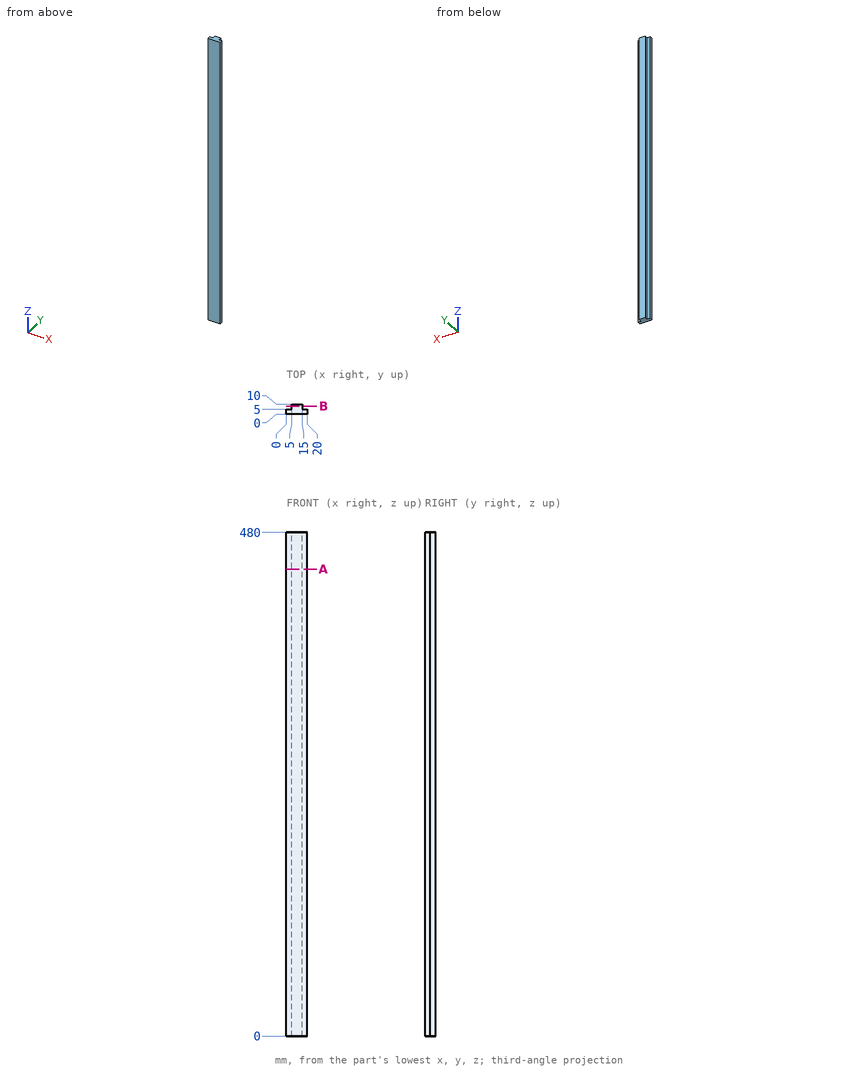
The drawing under review shows one solid part. Ordinate dimensions are in mm from its lowest x, y, z. Give positions to 0.01 mm unless a question says otherwise; leave off trailing zeros. Order: outer loops, then holes, each group sorted by start corner. A loop starts at its lowest first (then second) coordinate and runs counter-clockwise, first axis right, second up. Notation, with made-up numbers: (26.25, -14.5) - (55.25, -14.5) arc R28 cw to (55.25, 8.5) - close; hole circle Ø10 at (59.25, 50). An arc over 180 degrees is marked (long way). Answer as a JSON object with one key per item and string values. Group by question number.
Item 1: Wall thickness on line 1 along Y through (x, z) = (15.75, 396); line 2 along X through (y, z) = (5.5, 82.5): over which ranges is each line inside the solid? List them lowest first.
Item 2: Take a section at B-B on y = 8. Give the boundary of the cut face in (x, z).
Item 3: Clearance check with flat-ended pins moving along their axes: pin 1 Ø3 at (y, z) = (2.5, 319) entering from -X; pin 2 Ø1.5 at (y, z) = (8, 257) entering from -X; pin 3 Ø1.5 at (y, z) = (7, 210.5) entering from +X; pin 4 Ø1.5 at (x, z) = (18.5, 348.5) entering from +Y. State where each tip first meets the part, or that it passes through.
Item 4: Take a section at A-A on z = 445. Give the boundary of the cut face in (x, y).
Reported:
{
 "1": {"line 1": "0 to 5", "line 2": "5 to 15"},
 "2": {"outline": "(5, 0) - (15, 0) - (15, 480) - (5, 480) - close"},
 "3": {"pin 1": "x = 0", "pin 2": "x = 5", "pin 3": "x = 15", "pin 4": "y = 5"},
 "4": {"outline": "(0, 0) - (20, 0) - (20, 5) - (15, 5) - (15, 10) - (5, 10) - (5, 5) - (0, 5) - close"}
}
